```python
from build123d import *

# Parameters (mm, degrees)
SKETCH2_R          = 5.5
CUT_EXTRUDE1_DEPTH = 85


with BuildPart() as part:
    # Sketch1 → Revolve1 (revolve)
    with BuildSketch(Plane.XY, mode=Mode.PRIVATE) as revolve1_sk:
        with BuildLine():
            Line((-357.644251927, 160.5), (-391.444251927, 160.5))
            ThreePointArc((-391.444251927, 160.5), (-392.151358708, 160.207106781), (-392.444251927, 159.5))
            Line((-392.444251927, 159.5), (-392.444251927, 131))
            Line((-392.444251927, 131), (-392.444251927, 75))
            Line((-392.444251927, 75), (-407.444251927, 75))
            Line((-407.444251927, 75), (-407.444251927, 131))
            Line((-407.444251927, 131), (-407.444251927, 170.5))
            ThreePointArc((-407.444251927, 170.5), (-405.979785833, 174.035533906), (-402.444251927, 175.5))
            Line((-402.444251927, 175.5), (-372.644251927, 175.5))
            ThreePointArc((-372.644251927, 175.5), (-369.108718021, 176.964466094), (-367.644251927, 180.5))
            Line((-367.644251927, 180.5), (-367.644251927, 205))
            Line((-367.644251927, 205), (-367.644251927, 230.5))
            Line((-367.644251927, 230.5), (-352.644251927, 230.5))
            Line((-352.644251927, 230.5), (-352.644251927, 205.5))
            Line((-352.644251927, 205.5), (-352.644251927, 165.5))
            ThreePointArc((-352.644251927, 165.5), (-354.108718021, 161.964466094), (-357.644251927, 160.5))
        make_face()
    revolve(revolve1_sk.sketch.rotate(Axis((0, 0, 0), (-1, 0, 0)), 90), axis=Axis((0, 0, 0), (-1, 0, 0)))

    # Sketch2 → Cut-Extrude1 (cut)
    with BuildSketch(Plane.ZY.offset(367.644251927)):
        with Locations((0, 210)):
            Circle(SKETCH2_R)
        with Locations((181.865334795, 105)):
            Circle(SKETCH2_R)
        with Locations((181.865334795, -105)):
            Circle(SKETCH2_R)
        with Locations((0, -210)):
            Circle(SKETCH2_R)
        with Locations((-181.865334795, -105)):
            Circle(SKETCH2_R)
        with Locations((-181.865334795, 105)):
            Circle(SKETCH2_R)
    extrude(amount=-CUT_EXTRUDE1_DEPTH, mode=Mode.SUBTRACT)


solid = part.part
```
Geometry check sheet. Reference: the model listing, model coordinates, mm. A direction names the side the tool comes from. Coordinates: 2 decimals unless noted, no trailing zeros. Order: outer loops, then holes, each group sorted by start corner. A loop starts at its lowest first (then second) coordinate and runs counter-clockwise, first axis right, second up. Notation, with made-up numbers: M -2,77.25 L 55,77.25 A30 cw 55,100.25 Z; hole C 81,71.5 d10. An arc over 180 degrees is marked long. One line per question, with ' | ' between items. Start each with the question number.
Item 1: Set-up check for faces 1 (the flat face through (-392.444, 33, -69)), 2 (the cylindrical face through (-387.336, -174.007, 22.847)), 3 (the cylindrical face through (-360.25, -100.36, 184.82)): record each of +Z, -Z, +X, -X, +Y, -Y from which the full face is reachable in a straight line by a thin tool's end or side.
Item 2: Material ranges on L1, parallel to X at y = -159, z = 14; L2, parallel to X at y = -143, z = 93.5; L3, parallel to Y at x = -382, z = 45, recorded low to high. Write a range as [from, to].
Item 3: Cross-section at B-B on z = 0. State how many separate pieces and enclosed holes the cut face has, then the cut area to 3 significant figures.
Item 4: Cross-section at A-A on y = 0. Enter the section's corners in (x, z).
Item 5: Cross-section at C-C on x = -382. Enter the section's corners in (y, z).
Item 6: Draft check along Y on faces 4 (the cylindrical face through (-360.039, 204.493, -106.362)), 5 (the cylindrical face through (-360.25, -104.76, -187.36)), 6 (the flat face through (-352.644, -121, -118)), 7 (the cylindrical face through (-374.78, 97.66, 127.37)). Enter one of: pulls with the +Y half, pulls with the -Y half, needs draft (parallel to the pull), parting line crosses it, or undercut.
Item 7: Gauge pin test, flat ends, axial feed: pin 1 (6 mm diameter, centred on x = -358.5, y = -41, fed in from +Z); pin 2 (3 mm diameter, centred on x = -378.5, z = -131, fed in from +Y); pin 3 (1 mm diameter, centred on x = -372.5, z = -112.5, fed in from -Y); pin 4 (9 mm diameter, centred on y = -105, z = -181.87, fed in from +X). Record the tip position at first contact, or that the pin passes through.
Findings:
1) face 1: +X | face 2: -X | face 3: +X, -X
2) L1: x = [-407.44, -392.44] | L2: x = [-407.43, -352.64] | L3: y = [-169.63, -154.06], [154.06, 169.63]
3) separate pieces: 4 | enclosed holes: 0 | area: 5,520 mm²
4) outline: M -407.44,-170.5 A5 ccw -402.44,-175.5 L -372.64,-175.5 A5 cw -367.64,-180.5 L -367.64,-230.5 L -352.64,-230.5 L -352.64,-165.5 A5 ccw -357.64,-160.5 L -391.44,-160.5 A1 cw -392.44,-159.5 L -392.44,-75 L -407.44,-75 Z; M -407.44,75 L -392.44,75 L -392.44,159.5 A1 cw -391.44,160.5 L -357.64,160.5 A5 ccw -352.64,165.5 L -352.64,230.5 L -367.64,230.5 L -367.64,180.5 A5 cw -372.64,175.5 L -402.44,175.5 A5 ccw -407.44,170.5 Z
5) outline: C 0,0 d351; hole C 0,0 d321
6) face 4: parting line crosses it | face 5: undercut | face 6: needs draft | face 7: undercut
7) pin 1: stops at z = 227.35 | pin 2: stops at y = 118.45 | pin 3: stops at y = -135.12 | pin 4: passes through
